Can you work these out from the model? Positions are in its coordinate system, mm. A direction names the side the tool comes from. Coordinates: 2 decimals unless noted, no trailing zeros. Order: outer loops, then holes, each group sorted by start corner. A loop starts at its lowest first (then second) coordinate and runs counter-clockwise, first axis right, second up.
```python
from build123d import *

# Parameters (mm, degrees)
SKETCH_1_W                = 30
SKETCH_1_H                = 310
EXTRUDE_1_DEPTH           = 15
HOLE_WIZARD_1_D           = 6.6
HOLE_WIZARD_1_CBORE_D     = 11
HOLE_WIZARD_1_CBORE_DEPTH = 6.8
FILLET_1_R                = 10


with BuildPart() as part:
    # 草图1 → 凸台-拉伸1 (new body)
    with BuildSketch(Plane.XY):
        Rectangle(SKETCH_1_W, SKETCH_1_H)
    extrude(amount=EXTRUDE_1_DEPTH)

    # 打孔尺寸(%根据)内六角圆柱头螺钉的类型1 (through all)
    with Locations(Plane(origin=(0, 0, 0), x_dir=(-1, 0, 0), z_dir=(0, 0, -1))):
        with Locations((0, 105), (0, -15), (0, -135)):
            CounterBoreHole(HOLE_WIZARD_1_D / 2, HOLE_WIZARD_1_CBORE_D / 2, HOLE_WIZARD_1_CBORE_DEPTH)

    # 圆角1
    fillet_1_edges = [part.edges().sort_by_distance(p)[0] for p in [
        (0, 155, 0),
    ]]
    fillet(fillet_1_edges, radius=FILLET_1_R)


solid = part.part
```
1. I'm going to push flat-ended pins straight in: pin 1 (10.5 mm diameter, centred on x = 0, y = 105, fed in from -Z); pin 2 (17.5 mm diameter, centred on x = 0, y = -135, fed in from -Z); pin 3 (6 mm diameter, centred on x = 0, y = -15, fed in from -Z). Where does each tip first touch, or does it pass through?
Completed:
pin 1: stops at z = 6.8
pin 2: stops at z = 0
pin 3: passes through
2. Imagine slicing it at C-C on z = 4.5. Please give me the cut outline in (x, y).
Completed:
outline: (-15, -155) - (15, -155) - (15, 153.35) - (-15, 153.35) - close; hole circle Ø11 at (0, -135); hole circle Ø11 at (0, -15); hole circle Ø11 at (0, 105)
3. Imagine slicing it at A-A on y = -135. Please give me the cut outline in (x, z).
Completed:
outline: (-15, 0) - (-5.5, 0) - (-5.5, 6.8) - (-3.3, 6.8) - (-3.3, 15) - (-15, 15) - close; (3.3, 6.8) - (5.5, 6.8) - (5.5, 0) - (15, 0) - (15, 15) - (3.3, 15) - close
4. Thinking about a two-plate mould opening in Y: for faces 1 (the cylindrical face through (0.21, 152.15, 3.01)), 2 (the flat face through (-15, -2, 7)), 3 (the cylindrical face through (1.774, 107.783, 10.957)), which applies, pulls with the +Y half, pulls with the -Y half, needs draft (parallel to the pull), parting line crosses it, or undercut?
Completed:
face 1: pulls with the +Y half
face 2: needs draft
face 3: undercut
5. Please list where these lines run through material, in increasing order: probe 1 along Y at (x, z) = (0, 12); probe 2 along Y at (x, z) = (0.75, 9.75); probe 3 along Z at (x, y) = (-3.25, -16).
Completed:
probe 1: y = -155 to -138.3, -131.7 to -18.3, -11.7 to 101.7, 108.3 to 155
probe 2: y = -155 to -138.21, -131.79 to -18.21, -11.79 to 101.79, 108.21 to 155
probe 3: z = 6.8 to 15
6. Imagine slicing it at B-B on x = 0. Give the number of separate pieces and of enclosed holes in the cut face, then the cut area to 3 significant figures.
Completed:
separate pieces: 4
enclosed holes: 0
area: 4,240 mm2
7. On a 3-axis mill with a long thin cutter (end or side, diameter ignored), from which of +Z, -Z, +X, -X, +Y, -Y can I reach the whole of each face in a straight line? I mean faces 4 (the cylindrical face through (0.716, -129.547, 3.352)), 5 (the flat face through (15, -2, 7)). Say none if no direction works.
Completed:
face 4: -Z
face 5: +Z, -Z, +X, +Y, -Y
